Check sheet for the drawn part. Datum: minimum x, y, z corner. Units: mm. Coordinates: 2 decimals unless noted, no trailing zeros. Order: outer loops, then holes, each group sorted by start corner. A loop starts at its lowest first (then second) coordinate and runs counter-clockwise, first axis right, second up.
Q1. Cross-section at D-D, the plane x = 34. Record the boundary of the cut face in (y, z).
Q2. Cross-section at C-C, the plane z = 3. Record the boundary of the cut face in (x, y), and give its area (3 significant figures).
Q3. Cross-section at A-A, the plane x = 70. Record the boundary of the cut face in (y, z), and give its area (3 significant figures).
Q4. Depth check by flat-ended pin: P1, Ø3, axis at x = 122, z = 15, coming from the -Y side; P2, Ø5, axis at y = 16.5, z = 21, coming from the +X side; P3, Ø14.5, axis at x = 70, y = 20, coming from the -Z side. Enter the tip coordinate at first touch or a pass-through.
Q5. Cross-section at B-B, the plane y = 20. Record the boundary of the cut face in (x, z).
Q6. Draft check along Y on the marked faces 1, 2 and 3. Enter one of: pulls with the +Y half, pulls with the -Y half, needs draft (parallel to the pull), parting line crosses it, or undercut.
Q7. Thickness scan on line 1 (Y direction, x = 70, z = 24); line 2 (Y direction, x = 70, z = 12.5); line 3 (Z direction, x = 79.5, y = 126.5). Record the ranges inside material, lowest first.
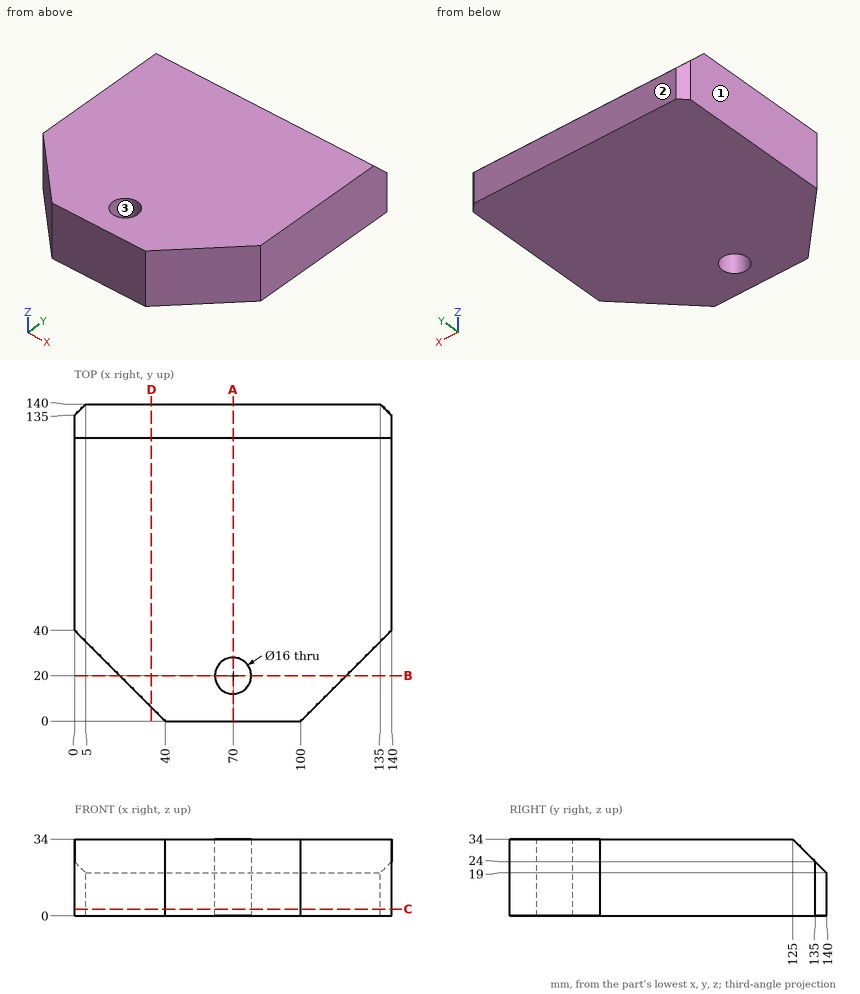
Check values:
1. outline: (6, 0) - (140, 0) - (140, 19) - (125, 34) - (6, 34) - close
2. outline: (0, 40) - (40, 0) - (100, 0) - (140, 40) - (140, 135) - (135, 140) - (5, 140) - (0, 135) - close; hole circle Ø16 at (70, 20)
2. area: 17,800 mm2
3. outline: (0, 0) - (12, 0) - (12, 34) - (0, 34) - close; (28, 0) - (140, 0) - (140, 19) - (125, 34) - (28, 34) - close
3. area: 4,100 mm2
4. P1: stops at y = 20.5
4. P2: stops at x = 119
4. P3: passes through
5. outline: (20, 0) - (62, 0) - (62, 34) - (20, 34) - close; (78, 0) - (120, 0) - (120, 34) - (78, 34) - close
6. face 1: needs draft
6. face 2: pulls with the +Y half
6. face 3: undercut
7. line 1: y = 0 to 12, 28 to 135
7. line 2: y = 0 to 12, 28 to 140
7. line 3: z = 0 to 32.5
